from build123d import *

# Parameters (mm, degrees)
BOSS_EXTRUDE1_DEPTH   = 12
SKETCH2_W             = 3
SKETCH2_H             = 20
CUT_EXTRUDE1_DEPTH    = 30.732137495
SKETCH3_R             = 1.5
CUT_EXTRUDE2_DEPTH    = 29.91366459
M6_TAPPED_HOLE1_D     = 5
M6_TAPPED_HOLE1_DEPTH = 6
M6_TAPPED_HOLE1_TIP   = 1.502151548


with BuildPart() as part:
    # Sketch1 → Boss-Extrude1 (new body)
    with BuildSketch(Plane.XY):
        with BuildLine():
            Line((-4, 0), (-4, 22))
            ThreePointArc((-4, 22), (0, 26), (4, 22))
            Line((4, 22), (4, 0))
            ThreePointArc((4, 0), (0, -4), (-4, 0))
        make_face()
    extrude(amount=BOSS_EXTRUDE1_DEPTH)

    # Sketch2 → Cut-Extrude1 (cut, through all)
    with BuildSketch(Plane.ZY.offset(4)):
        with Locations((6, 26)):
            Rectangle(SKETCH2_W, SKETCH2_H)
        with Locations((6, -4)):
            Rectangle(SKETCH2_W, SKETCH2_H)
    extrude(amount=-CUT_EXTRUDE1_DEPTH, mode=Mode.SUBTRACT)

    # Sketch3 → Cut-Extrude2 (cut, through all)
    with BuildSketch(Plane.XY.offset(12)):
        with Locations((0, 22)):
            Circle(SKETCH3_R)
        Circle(SKETCH3_R)
    extrude(amount=-CUT_EXTRUDE2_DEPTH, mode=Mode.SUBTRACT)

    # M6 Tapped Hole1
    with Locations(Plane(origin=(4, 11, 6), x_dir=(0, 0, 1), z_dir=(1, 0, 0))):
        with Locations((0, 0)):
            Hole(M6_TAPPED_HOLE1_D / 2, depth=M6_TAPPED_HOLE1_DEPTH)
            with Locations((0, 0, -(M6_TAPPED_HOLE1_DEPTH + M6_TAPPED_HOLE1_TIP / 2))):  # 118° drill point
                Cone(0, M6_TAPPED_HOLE1_D / 2, M6_TAPPED_HOLE1_TIP, mode=Mode.SUBTRACT)


solid = part.part
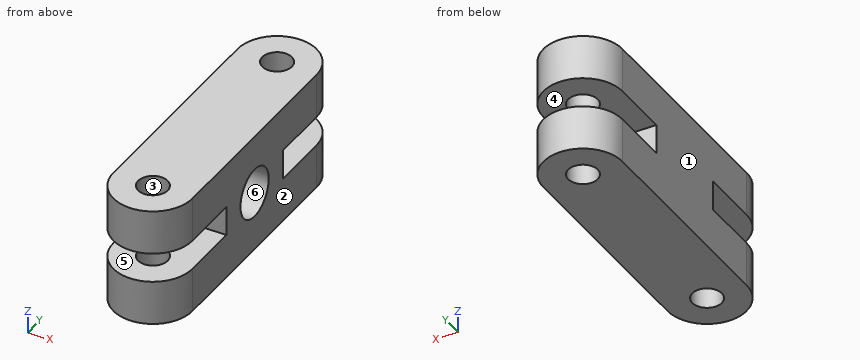
Verification items for the finished model (mm, model axes). Face numbers are marked on the shaded views. A direction names the side the tool comes from. Give positions to 0.01 mm unless a question says otherwise; leave off trailing zeros. Loops run counter-clockwise (first coordinate to the right, second up) from the corner with the lowest first, then second, coordinate; pieces in that order, holes last.
1. Release check for a two-part mould opening along X. For the marked faces 1, 2 and 3 record: +X half, -X half, draft (parallel to the pull), parting line (faces both ways), or undercut.
Derived:
face 1: -X half
face 2: +X half
face 3: undercut
2. Cross-section at D-D on x = 2.75. Record the cut outline in (y, z), and give its area (3 significant figures).
Derived:
outline: (-2.9, 0) - (24.9, 0) - (24.9, 4.5) - (16, 4.5) - (16, 7.5) - (24.9, 7.5) - (24.9, 12) - (-2.9, 12) - (-2.9, 7.5) - (6, 7.5) - (6, 4.5) - (-2.9, 4.5) - close; hole circle Ø5 at (11, 6)
area: 261 mm2
3. Tool access check on the marked faces 4, 5 and 6. Record the directions out of +Z, -Z, +X, -X, +Y, -Y that give a thin tool (end or side, any length) a straight path to the whole face; none if there is none.
Derived:
face 4: +X, -X, +Y
face 5: +X, -X, -Y
face 6: +X
4. Material ranges on probe 1 along Y at (x, z) = (0, 9.5); probe 2 along Z at (x, y) = (-3.5, 23.5); probe 3 along Z at (x, y) = (2.8, 11), recorded low to high.
Derived:
probe 1: y = -4 to -1.5, 1.5 to 20.5, 23.5 to 26
probe 2: z = 0 to 4.5, 7.5 to 12
probe 3: z = 0 to 3.5, 8.5 to 12
5. Cross-section at C-C on x = -2.75. Record the cut outline in (y, z).
Derived:
outline: (-2.9, 0) - (24.9, 0) - (24.9, 4.5) - (16, 4.5) - (16, 7.5) - (24.9, 7.5) - (24.9, 12) - (-2.9, 12) - (-2.9, 7.5) - (6, 7.5) - (6, 4.5) - (-2.9, 4.5) - close; hole circle Ø2.5 at (11, 6)
6. Go/stop test with flat-tipped pins: P1, Ø1.5, axis at x = 0.5, z = 5.5, coming from the -Y side; P2, Ø4, axis at x = -3, z = 9, coming from the -Y side; P3, Ø4.5, axis at y = 11, z = 6, coming from the +X side. Record where each tip stops, or that it passes through.
Derived:
P1: stops at y = 6
P2: stops at y = -3.87
P3: stops at x = -2.15
7. Cross-section at A-A on x = 0. Count the separate pieces of the cut face and the enclosed holes in it, and give its area (3 significant figures).
Derived:
separate pieces: 5
enclosed holes: 1
area: 226 mm2
8. Cross-section at B-B on z = 2. Record the cut outline in (x, y), and give its area (3 significant figures).
Derived:
outline: (-4, 0) arc R4 ccw to (4, 0) - (4, 22) arc R4 ccw to (-4, 22) - close; hole circle Ø3 at (0, 0); hole circle Ø3 at (0, 22)
area: 212 mm2
